```python
from build123d import *

# Parameters (mm, degrees)
SKETCH1_R           = 5.5
BOSS_EXTRUDE1_DEPTH = 24
SKETCH2_R           = 9
BOSS_EXTRUDE2_DEPTH = 12
CUT_EXTRUDE1_DEPTH  = 6


with BuildPart() as part:
    # Sketch1 → Boss-Extrude1 (new body)
    with BuildSketch(Plane.XY):
        Circle(SKETCH1_R)
    extrude(amount=BOSS_EXTRUDE1_DEPTH)

    # Sketch2 → Boss-Extrude2 (add)
    with BuildSketch(Plane.XY.offset(24)):
        Circle(SKETCH2_R)
    extrude(amount=BOSS_EXTRUDE2_DEPTH)

    # Sketch3 → Cut-Extrude1 (cut)
    with BuildSketch(Plane.XY.offset(36)):
        Polygon((0, 5.773502692), (-5, 2.886751346), (-5, -2.886751346), (0, -5.773502692), (5, -2.886751346), (5, 2.886751346), align=None)
    extrude(amount=-CUT_EXTRUDE1_DEPTH, mode=Mode.SUBTRACT)


solid = part.part
```
The model under review builds one solid part; all positions refer to its coordinate system, in mm. A direction names the side the tool comes from. Give positions to 0.01 mm unless a question says otherwise; leave off trailing zeros. Write each loop counter-clockwise with the first axis right and the second up, starting at its lowest first coordinate (ties: lowest second). Pieces come first, ordered by that corner, then holes. Notation, with made-up numbers: (-19, 14.5) -> (21, 14.5) arc R18 cw to (21, 39.5) -> close; hole circle Ø4 at (6, 48.25). An arc over 180 degrees is marked (long way). Answer in a Markdown table with one row per item.
1) Add section B-B on y = 0. State the section outline as (x, z) points.
Worked answers:
| item | result |
|---|---|
| outline | (-9, 24) -> (-5.5, 24) -> (-5.5, 0) -> (5.5, 0) -> (5.5, 24) -> (9, 24) -> (9, 36) -> (5, 36) -> (5, 30) -> (-5, 30) -> (-5, 36) -> (-9, 36) -> close |
2) Add section D-D on z = 17. State the section outline as (x, y) points.
Worked answers:
| item | result |
|---|---|
| outline | circle Ø11 at (0, 0) |
3) Clearance check with flat-ended pins moving along their axes: P1, Ø5, axis at y = 0, z = 13.5, coming from the -X side; P2, Ø3, axis at x = 2, y = 2, coming from the +Z side; P3, Ø5, axis at y = 6.5, z = 10.5, coming from the -X side. State where each tip first meets the part, or that it passes through.
Worked answers:
| item | result |
|---|---|
| P1 | x = -5.5 |
| P2 | z = 30 |
| P3 | x = -3.77 |
4) Mouldability with a two-part tool opening along Y and no side actions: class faces 4 (the cylindrical face through (-1.19, -5.37, 11.83)), 5 (the flat face through (4, -4, 36)), 6 (the flat face through (5, 0, 33)) as +Y half, -Y half, draft (parallel to the pull), parting line (faces both ways), or undercut.
Worked answers:
| item | result |
|---|---|
| face 4 | parting line |
| face 5 | draft |
| face 6 | undercut |
5) Add section A-A on z = 32.5. State the section outline as (x, y) points, plus the area to 3 significant figures.
Worked answers:
| item | result |
|---|---|
| outline | circle Ø18 at (0, 0); hole (-5, -2.89) -> (0, -5.77) -> (5, -2.89) -> (5, 2.89) -> (0, 5.77) -> (-5, 2.89) -> close |
| area | 168 mm² |
6) For L1, parallel to X at y = 0.25, z = 32.5; L2, parallel to Z at x = -6, y = 5.5; L3, parallel to Z at x = 4, y = -0.5, list the stretches that pass through material, from the lowest coordinate up. Write a range as [from, to].
Worked answers:
| item | result |
|---|---|
| L1 | [-9, -5], [5, 9] |
| L2 | [24, 36] |
| L3 | [0, 30] |
7) Add section C-C on x = 2.5. State the section outline as (y, z) points, plus the area to 3 significant figures.
Worked answers:
| item | result |
|---|---|
| outline | (-8.65, 24) -> (-4.9, 24) -> (-4.9, 0) -> (4.9, 0) -> (4.9, 24) -> (8.65, 24) -> (8.65, 36) -> (4.33, 36) -> (4.33, 30) -> (-4.33, 30) -> (-4.33, 36) -> (-8.65, 36) -> close |
| area | 391 mm² |
8) Tool access review of faces 1 (the flat face through (2.535, 4.31, 33.042)), 2 (the flat face through (-4, -4, 24)), 3 (the cylindrical face through (-1.172, 8.923, 29.916)): name each direction out of +Z, -Z, +X, -X, +Y, -Y from which nothing blocks a thin tool from reaching the whole face with its end or side.
Worked answers:
| item | result |
|---|---|
| face 1 | +Z |
| face 2 | -Z |
| face 3 | +Z, -Z |
